from build123d import *

# Parameters (mm, degrees)
BOSS_EXTRUDE_1_DEPTH = 100
CUT_EXTRUDE_1_DEPTH  = 266.035846632
SKETCH_3_R           = 42.6
SKETCH_3_R_2         = 5
CUT_EXTRUDE_2_DEPTH  = 274.50319925
FILLET_1_R           = 30
FILLET_2_R           = 10


with BuildPart() as part:
    # Sketch 1 → Boss-Extrude 1 (new, symmetric)
    with BuildSketch(Plane.XY):
        Polygon((-60, 0), (0, 0), (0, 250), (-12, 250), (-12, 12), (-60, 12), align=None)
    extrude(amount=BOSS_EXTRUDE_1_DEPTH, both=True)

    # Sketch 2 → Cut-Extrude 1 (cut, through all)
    with BuildSketch(Plane(origin=(0, 12, 0), x_dir=(1, 0, 0), z_dir=(0, 1, 0))):
        with BuildLine():
            Line((-42.5, 67.5), (-42.5, 72.5))
            ThreePointArc((-42.5, 72.5), (-37, 78), (-31.5, 72.5))
            Line((-31.5, 72.5), (-31.5, 67.5))
            ThreePointArc((-31.5, 67.5), (-37, 62), (-42.5, 67.5))
        make_face()
        with BuildLine():
            Line((-42.5, -67.5), (-42.5, -72.5))
            ThreePointArc((-42.5, -72.5), (-37, -78), (-31.5, -72.5))
            Line((-31.5, -72.5), (-31.5, -67.5))
            ThreePointArc((-31.5, -67.5), (-37, -62), (-42.5, -67.5))
        make_face()
    extrude(amount=-CUT_EXTRUDE_1_DEPTH, mode=Mode.SUBTRACT)

    # Sketch 3 → Cut-Extrude 2 (cut, through all)
    with BuildSketch(Plane.ZY.offset(12)):
        with Locations(Location((0, 147, 0), (0, 0, 270))):
            Circle(SKETCH_3_R)
        with Locations(Location((0, 217, 0), (0, 0, 270))):
            Circle(SKETCH_3_R_2)
        with Locations(Location((0, 77, 0), (0, 0, 90))):
            Circle(SKETCH_3_R_2)
    extrude(amount=-CUT_EXTRUDE_2_DEPTH, mode=Mode.SUBTRACT)

    # Fillet 1
    fillet_1_edges = [part.edges().sort_by_distance(p)[0] for p in [
        (-6, 250, 100),
        (-6, 250, -100),
    ]]
    fillet(fillet_1_edges, radius=FILLET_1_R)

    # Fillet 2
    fillet_2_edges = [part.edges().sort_by_distance(p)[0] for p in [
        (-60, 6, 100),
        (-60, 6, -100),
    ]]
    fillet(fillet_2_edges, radius=FILLET_2_R)


solid = part.part
Work out the finished part from the listing and answer in its coordinate system (mm). A direction names the side the tool comes from. Coordinates: 2 decimals unless noted, no trailing zeros. Write each loop counter-clockwise with the first axis right and the second up, starting at its lowest first coordinate (ties: lowest second). Pieces come first, ordered by that corner, then holes. Notation, with made-up numbers: M -34,29.25 L -10,29.25 A31 cw -10,55.25 Z; hole C 55.5,-3 d2. An arc over 180 degrees is marked long. Use one line per item in the form item = value. Start each with the question number.
1. The part is cut by section B-B (x = -4). Give the vertices of the cut face in (y, z), plus the area to 3 significant figures.
2. Straight lines are drawn through the part: probe 1 along Z at (x, y) = (-7, 217); probe 2 along X at (y, z) = (84, -77.5); probe 3 along Y at (x, z) = (-31, 60.5). For each, find the intervals that lie inside material, in ascending order. Write a range as from..to.
3. The part is cut by section C-C (z = -30). Give the vertices of the cut face in (x, y) (3 decimals).
4. The part is cut by section A-A (y = 77). Give the vertices of the cut face in (x, z), plus the area to 3 significant figures.
5. The part is cut by section D-D (x = -15.5). Give the vertices of the cut face in (y, z), plus the area to 3 significant figures.
6. The mould has two halves that part along Y. Classify faces 4 (the face through (-30, 0, 1)), 5 (the face through (-6.08, 189.56, 1.87)), 6 (the face through (-6.08, 212.23, 1.5)), 7 (the face through (-31.5, 6, -70)): released by +Y, released by -Y, zero draft, split by the parting line, or undercut.
7. Each of these flat-tipped pins is pushed along its axis until it touches: P1, Ø1, axis at y = 72, z = -38.5, coming from the -X side; P2, Ø11.5, axis at y = 217, z = 0, coming from the +X side; P3, Ø14.5, axis at x = -36.5, z = -43.5, coming from the +Y side. Where does it stop, or does it pass through?
8. A tool of negligible diameter and unlimited length cuts with its end or side. For faces 1 (the face through (-6.084, 240.979, 91.445)), 2 (the face through (-36, 12, 1)), 3 (the face through (-42.5, 6, 70)), from which of +Z, -Z, +X, -X, +Y, -Y can it reach the whole face along a straight path? Write none if from no direction.
Evaluation:
q1.outline = M 0,-100 L 220,-100 A30 ccw 250,-70 L 250,70 A30 ccw 220,100 L 0,100 Z; hole C 77,0 d10; hole C 147,0 d85.2; hole C 217,0 d10
q1.area = 43,800 mm^2
q2.probe_1 = -100..-5, 5..100
q2.probe_2 = -12..0
q2.probe_3 = 0..12
q3.outline = M -60,0 L 0,0 L 0,116.755 L -12,116.755 L -12,12 L -60,12 Z; M -12,177.245 L 0,177.245 L 0,250 L -12,250 Z
q4.outline = M -12,-100 L 0,-100 L 0,-5 L -12,-5 Z; M -12,5 L 0,5 L 0,100 L -12,100 Z
q4.area = 2,280 mm^2
q5.outline = M 0,-100 L 12,-100 L 12,100 L 0,100 Z
q5.area = 2,400 mm^2
q6.face_4 = released by -Y
q6.face_5 = undercut
q6.face_6 = undercut
q6.face_7 = zero draft
q7.P1 = -12
q7.P2 = 0
q7.P3 = 12
q8.face_1 = +Z, +X, -X, +Y
q8.face_2 = +Z, -Z, -X, +Y
q8.face_3 = +Y, -Y
